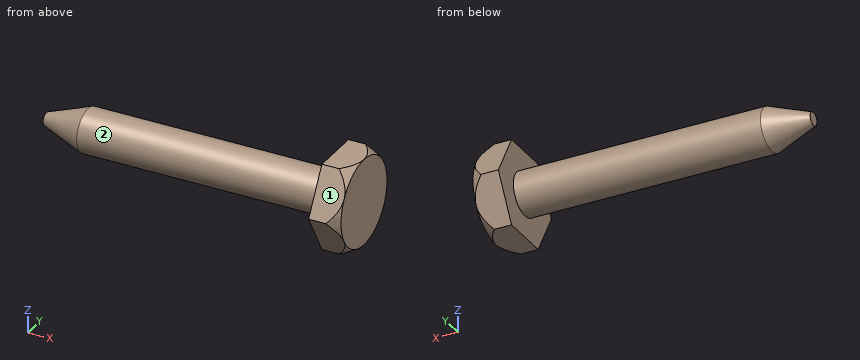
```python
from build123d import *

# Parameters (mm, degrees)
BOSS_EXTRUDE1_DEPTH = 4
SKETCH2_OUTSIDE_W   = 22.372
SKETCH2_OUTSIDE_H   = 24.228
SKETCH2_OUTSIDE_R   = 6
CUT_EXTRUDE1_DEPTH  = 4
CUT_EXTRUDE1_DRAFT  = -30


with BuildPart() as part:
    # Sketch1 → Boss-Extrude1 (new body)
    with BuildSketch(Plane(origin=(0, 0, 0), x_dir=(0, 0, -1), z_dir=(1, 0, 0))):
        Polygon((0, -6.92820323), (6, -3.464101615), (6, 3.464101615), (0, 6.92820323), (-6, 3.464101615), (-6, -3.464101615), align=None)
    extrude(amount=BOSS_EXTRUDE1_DEPTH)


with BuildPart() as cut_extrude1_tool:
    # Sketch2 outside → Cut-Extrude1 (with draft: the straight prism first)
    with BuildSketch(Plane(origin=(4, 0, 0), x_dir=(0, 0, -1), z_dir=(1, 0, 0))):
        Rectangle(SKETCH2_OUTSIDE_W, SKETCH2_OUTSIDE_H)
        Circle(SKETCH2_OUTSIDE_R, mode=Mode.SUBTRACT)
    extrude(amount=-CUT_EXTRUDE1_DEPTH)
    # Cut-Extrude1: the draft: its side faces are tilted about the plane it starts from
    cut_extrude1_sides = [cut_extrude1_tool.faces().sort_by_distance(p)[0] for p in [
        (2, -12.114, 0),
        (2, 0, -11.186),
        (2, 12.114, 0),
        (2, 0, 11.186),
        (2, 0, 6),
    ]]
    draft(cut_extrude1_sides, Plane(origin=(4, 0, 0), x_dir=(0, 0, -1), z_dir=(1, 0, 0)), CUT_EXTRUDE1_DRAFT)


with BuildPart() as part_1:
    add(part.part)

    # Cut-Extrude1: cut by cut_extrude1_tool
    add(cut_extrude1_tool.part, mode=Mode.SUBTRACT)

    # Sketch3 → Revolve1 (revolve)
    with BuildSketch(Plane.XY, mode=Mode.PRIVATE) as revolve1_sk:
        Polygon((0, 3), (0, 0), (-40, 0), (-40, 0.9), (-34.230297419, 3), align=None)
    revolve(revolve1_sk.sketch.rotate(Axis((-29.866000922, 0, 0), (1, 0, 0)), 90), axis=Axis((-29.866000922, 0, 0), (1, 0, 0)))


solid = part_1.part
```
Geometry: final body of the model. Coordinates: model frame, mm. Face numbers are marked on the shaded views. A direction names the side the tool comes from. Coordinates: 2 decimals unless noted, no trailing zeros. Loops run counter-clockwise (first coordinate to the right, second up) from the corner with the lowest first, then second, coordinate; pieces in that order, holes last. Notation, with made-up numbers: M 30.25,56.5 L 65.25,56.5 A29 cw 65.25,77.5 Z; hole C -11.5,-12.75 d4. An arc over 180 degrees is marked long. Put each result on its own line as item: value.
(1) First-contact query: pin 1 (8 mm diameter, centred on x = -30, y = 4, fed in from -Z); pin 2 (6 mm diameter, centred on x = -33, y = -5.5, fed in from +Z); pin 3 (1.5 mm diameter, centred on x = -8.5, z = -1.5, fed in from +Y). Flat tips, straight axial feed; report the tip coordinate or a pass-through.
Answer sheet:
pin 1: stops at z = -3
pin 2: stops at z = 1.66
pin 3: stops at y = 2.9
(2) Cut plane A-A on x = -2. Return the cut outline in (y, z), then the cut area to 3 significant figures.
Answer sheet:
outline: C 0,0 d6
area: 28.3 mm^2
(3) Access query for the marked faces 1 and 2. Directions: +Z, -Z, +X, -X, +Y, -Y. A direction counts if a zero-diameter tool reaches every point of the face in a straight line with its end or side. Return the directions, or none.
Answer sheet:
face 1: +Z, +X, -X, -Y
face 2: -X
(4) Material intervals for probe 1 along X at (y, z) = (-4, -0.25); probe 2 along Z at (x, y) = (-4.5, -0.75); probe 3 along Y at (x, z) = (-5, -1.5), sorted ascending.
Answer sheet:
probe 1: x = 0 to 4
probe 2: z = -2.9 to 2.9
probe 3: y = -2.6 to 2.6
